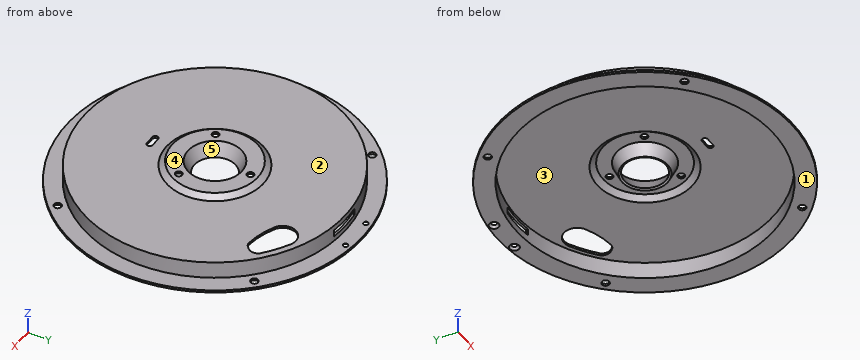
```python
from build123d import *

# Parameters (mm, degrees)
CUT_EXTRUDE1_DEPTH                                   = 45
CUT_EXTRUDE2_DEPTH                                   = 10
SKETCH5_W                                            = 30
SKETCH5_H                                            = 6
CUT_EXTRUDE3_DEPTH                                   = 32
HOLE_SIZE_BY_CROSS_RECESS_COUNTERSUNK_SE_D           = 3.7
HOLE_SIZE_BY_CROSS_RECESS_COUNTERSUNK_SE_CSINK_D     = 8.2
HOLE_SIZE_BY_CROSS_RECESS_COUNTERSUNK_SE_CSINK_ANGLE = 90
SKETCH8_R                                            = 3.25
CUT_EXTRUDE4_DEPTH                                   = 186.04323819
CIRPATTERN1_COUNT                                    = 4
SKETCH9_R                                            = 3
CUT_EXTRUDE5_DEPTH                                   = 28
CIRPATTERN2_COUNT                                    = 3


with BuildPart() as part:
    # Sketch1 → Revolve1 (revolve)
    with BuildSketch(Plane(origin=(0, 0, 0), x_dir=(1, 0, 0), z_dir=(0, 1, 0)), mode=Mode.PRIVATE) as revolve1_sk:
        Polygon((-115, 15), (-130, 15), (-130, 17), (-113, 17), (-113, 2), (-67.400598844, 2), (-42, 2), (-37, -2), (-25, -2), (-20, 8.5), (-18.194278962, 7.640132839), (-23.737199362, -4), (-37.701562119, -4), (-42.701562119, 0), (-115, 0), align=None)
    revolve(revolve1_sk.sketch.rotate(Axis((0, 0, 0), (0, 0, -1)), 180), axis=Axis((0, 0, 0), (0, 0, -1)))

    # Sketch3 → Cut-Extrude1 (cut)
    with BuildSketch(Plane(origin=(0, 0, -17), x_dir=(-1, 0, 0), z_dir=(0, 0, -1))):
        with BuildLine():
            Line((-69.977392836, 70.947139279), (-71.467016668, 72.43676311))
            ThreePointArc((-71.467016668, 72.43676311), (-73.65767572, 78.041003905), (-71.024689008, 83.451538346))
            ThreePointArc((-71.024689008, 83.451538346), (-61.250096658, 90.868538892), (-50.7076021, 97.146306107))
            ThreePointArc((-50.7076021, 97.146306107), (-34.862231231, 92.134081811), (-39.938869953, 76.309230795))
            ThreePointArc((-39.938869953, 76.309230795), (-52.260986787, 71.486832981), (-65.295075938, 69.205911249))
            ThreePointArc((-65.295075938, 69.205911249), (-67.826068353, 69.566044861), (-69.977392836, 70.947139279))
        make_face()
    extrude(amount=-CUT_EXTRUDE1_DEPTH, mode=Mode.SUBTRACT)

    # Sketch4 → Cut-Extrude2 (cut)
    with BuildSketch(Plane(origin=(0, 0, -2), x_dir=(-1, 0, 0), z_dir=(0, 0, -1))):
        with BuildLine():
            Line((-4, -52.5), (4, -52.5))
            ThreePointArc((4, -52.5), (6.5, -55), (4, -57.5))
            Line((4, -57.5), (-4, -57.5))
            ThreePointArc((-4, -57.5), (-6.5, -55), (-4, -52.5))
        make_face()
    extrude(amount=-CUT_EXTRUDE2_DEPTH, mode=Mode.SUBTRACT)

    # Sketch5 → Cut-Extrude3 (cut)
    with BuildSketch(Plane(origin=(0, 140, 0), x_dir=(1, 0, 0), z_dir=(0, 1, 0))):
        with Locations((0, 7.5)):
            Rectangle(SKETCH5_W, SKETCH5_H)
    extrude(amount=-CUT_EXTRUDE3_DEPTH, mode=Mode.SUBTRACT)

    # Hole size by cross-recess countersunk self-tapping screw type1 (through all)
    with Locations(Plane(origin=(15, 124, -17), x_dir=(-1, 0, 0), z_dir=(0, 0, -1))):
        with Locations((0, 0), (30, 0)):
            CounterSinkHole(HOLE_SIZE_BY_CROSS_RECESS_COUNTERSUNK_SE_D / 2, HOLE_SIZE_BY_CROSS_RECESS_COUNTERSUNK_SE_CSINK_D / 2, counter_sink_angle=HOLE_SIZE_BY_CROSS_RECESS_COUNTERSUNK_SE_CSINK_ANGLE)

    # Sketch8 → Cut-Extrude4 (cut, through all)
    with BuildSketch(Plane(origin=(0, 0, -17), x_dir=(-1, 0, 0), z_dir=(0, 0, -1))):
        with Locations((86.620580695, 86.620580695)):
            Circle(SKETCH8_R)
    cut_extrude4 = extrude(amount=-CUT_EXTRUDE4_DEPTH, mode=Mode.SUBTRACT)

    # CirPattern1: Cut-Extrude4 ×4 about axis
    cirpattern1_axis = Axis((0, 0, 0), (0, 0, 1))
    for i in range(1, CIRPATTERN1_COUNT):
        add(cut_extrude4.rotate(cirpattern1_axis, i * 360 / CIRPATTERN1_COUNT), mode=Mode.SUBTRACT)

    # Sketch9 → Cut-Extrude5 (cut)
    with BuildSketch(Plane(origin=(0, 0, 2), x_dir=(-1, 0, 0), z_dir=(0, 0, -1))):
        with Locations((0, 31.25)):
            Circle(SKETCH9_R)
    cut_extrude5 = extrude(amount=-CUT_EXTRUDE5_DEPTH, mode=Mode.SUBTRACT)

    # CirPattern2: Cut-Extrude5 ×3 about axis
    cirpattern2_axis = Axis((0, 0, 0), (0, 0, 1))
    for i in range(1, CIRPATTERN2_COUNT):
        add(cut_extrude5.rotate(cirpattern2_axis, i * 360 / CIRPATTERN2_COUNT), mode=Mode.SUBTRACT)


solid = part.part
```
Could you check a few things on this model? Use its own coordinates, in mm. Face numbers are marked on the shaded views. A direction names the side the tool comes from. Round coordinates to 2 decimals unless told otherwise and drop trailing zeros. Write each loop counter-clockwise with the first axis right and the second up, starting at its lowest first coordinate (ties: lowest second). Pieces come first, ordered by that corner, then holes. Notation, with made-up numbers: M 51,53.5 L 99,53.5 A26 ccw 99,74.5 Z; hole C 6,38.25 d6. An arc over 180 degrees is marked long. Answer in a Markdown table with one row per item. Add a question column.
Q1. Imagine slicing it at A-A (y = 0). Please give me the cut outline in (x, z).
Q2. If I drill on line 1 (X direction, y = -1, z = -10.75); line 2 (X direction, y = 3, z = -1.25); line 3 (Z direction, x = -110.5, y = -53), over which ranges is the centre line in solid material (lowest first)? Write a range as from..to.
Q3. On a 3-axis mill with a long thin cutter (end or side, diameter ignored), from which of +Z, -Z, +X, -X, +Y, -Y can I reach the whole of each face in a straight line? I mean the marked faces 1, 2 and 3. Say none if no direction works.
Q4. Imagine slicing it at C-C (x = -108). Please give me the cut outline in (y, z).
Q5. Imagine slicing it at D-D (y = -75.5). Please give me the cut outline in (x, z), then the cut area to 3 significant figures.
Q6. Imagine slicing it at B-B (y = 124). Please give me the cut outline in (x, z), then the cut area to 3 significant figures.
Q7. If we mould it in two halves opening along Y, with no side actions, what happens to the marked faces 4 and 5? For each: +Y half, -Y half, draft (parallel to the pull), parting line (faces both ways), or undercut.
Q8. Will these pins go through, and if not, where does the flat tip stop? pin 1 Ø1 at (y, z) = (-80.5, -7.5) entering from +X; pin 2 Ø10 at (x, z) = (20.5, 0) entering from -Y; pin 3 Ø6 at (y, z) = (95.5, -0.5) entering from +X; pin 4 Ø10.5 at (x, y) = (86.62, 86.62) entering from -Z.
Values:
| question | item | result |
|---|---|---|
| 1 | outline | M -130,-17 L -113,-17 L -113,-2 L -42,-2 L -37,2 L -25,2 L -20,-8.5 L -18.19,-7.64 L -23.74,4 L -37.7,4 L -42.7,0 L -115,0 L -115,-15 L -130,-15 Z; M 18.19,-7.64 L 20,-8.5 L 25,2 L 37,2 L 42,-2 L 113,-2 L 113,-17 L 130,-17 L 130,-15 L 115,-15 L 115,0 L 42.7,0 L 37.7,4 L 23.74,4 Z |
| 2 | line 1 | -115..-113, 113..115 |
| 2 | line 2 | -114.96..-40.95, -23.26..-21.02, 21.02..23.26, 40.95..114.96 |
| 2 | line 3 | -17..-15 |
| 3 | face 1 | -Z, +X, -X, +Y, -Y |
| 3 | face 2 | +Z |
| 3 | face 3 | -Z |
| 4 | outline | M -72.36,-17 L -33.24,-17 L -33.24,-2 L 33.24,-2 L 33.24,-17 L 72.36,-17 L 72.36,-15 L 39.51,-15 L 39.51,0 L -39.51,0 L -39.51,-15 L -72.36,-15 Z |
| 5 | outline | M -105.83,-17 L -84.08,-17 L -84.08,-2 L 84.08,-2 L 84.08,-17 L 105.83,-17 L 105.83,-15 L 86.75,-15 L 86.75,0 L -86.75,0 L -86.75,-15 L -105.83,-15 Z |
| 5 | area | 503 mm^2 |
| 6 | outline | M -39.04,-17 L -19.1,-17 L -17.1,-15 L -39.04,-15 Z; M -12.9,-15 L -10.9,-17 L 10.9,-17 L 12.9,-15 Z; M 17.1,-15 L 19.1,-17 L 39.04,-17 L 39.04,-15 Z |
| 6 | area | 131 mm^2 |
| 7 | face 4 | draft |
| 7 | face 5 | undercut |
| 8 | pin 1 | x = 82.61 |
| 8 | pin 2 | y = -113.95 |
| 8 | pin 3 | x = 68.33 |
| 8 | pin 4 | z = -17 |
